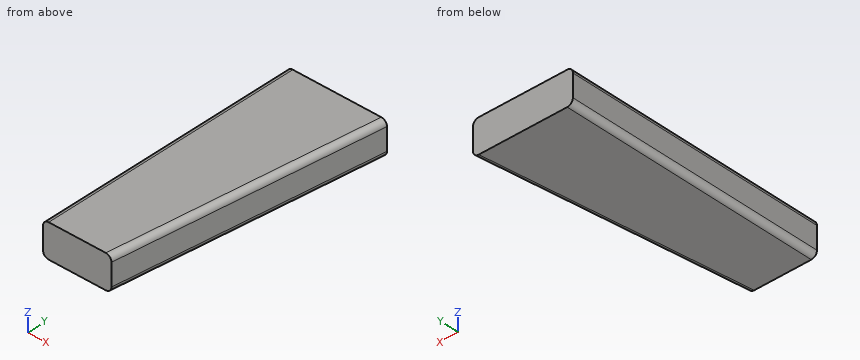
```python
from build123d import *

# Parameters (mm, degrees)
BOSS_EXTRUDE1_DEPTH = 118
FILLET1_R           = 20


with BuildPart() as part:
    # Sketch1 → Boss-Extrude1 (new body)
    with BuildSketch(Plane.XY):
        Polygon((0, 0), (240, 0), (350, 923), (0, 923), align=None)
    extrude(amount=BOSS_EXTRUDE1_DEPTH)

    # Fillet1
    fillet1_edges = [part.edges().sort_by_distance(p)[0] for p in [
        (295, 461.5, 118),
        (0, 461.5, 118),
        (295, 461.5, 0),
        (0, 461.5, 0),
    ]]
    fillet(fillet1_edges, radius=FILLET1_R)


solid = part.part
```
Verification items for the finished model (mm, model axes). Give positions to 0.01 mm unless a question says otherwise; leave off trailing zeros. Loops run counter-clockwise (first coordinate to the right, second up) from the corner with the lowest first, then second, coordinate; pieces in that order, holes last.
1. Go/stop test with flat-tipped pins: pin 1 Ø2 at (y, z) = (767, 76) entering from +X; pin 2 Ø3 at (y, z) = (371, 34.5) entering from +X. Record where each tip stops, or that it passes through.
2. Section check A-A, the plane z = 53. Enter the section's corners in (x, y), then the cut area to 3 significant figures.
3. Thickness scan on line 1 (X direction, y = 331, z = 80); line 2 (Z direction, x = 278, y = 355); line 3 (X direction, y = 637, z = 68). Record the ranges inside material, lowest first.
Geometry says:
1. pin 1: stops at x = 331.53
1. pin 2: stops at x = 284.39
2. outline: (0, 0) - (240, 0) - (350, 923) - (0, 923) - close
2. area: 272,000 mm2
3. line 1: x = 0 to 279.45
3. line 2: z = 7.64 to 110.36
3. line 3: x = 0 to 315.92
